Could you check a few things on this model? Use its own coordinates, in mm. Face numbers are marked on the shaded views. A direction names the side the tool comes from. Give positions to 0.01 mm unless a question says otherwise; leave off trailing zeros. Loops run counter-clockwise (first coordinate to the right, second up) from the corner with the lowest first, then second, coordinate; pieces in that order, holes last. Notation, with made-up numbers: (79, -27) -> (105, -27) arc R33 ccw to (105, 1) -> close; hole circle Ø6 at (-5, 69.25). An arc over 180 degrees is marked (long way). Write each question's results on one line, items separated by ' | '. Start each with the question number.
Q1. We'd pull the mould along Z, two halves only. Please class the marked faces 3, 4 and 5: released by +Z, released by -Z, zero draft, split by the parting line, or undercut.
Q2. If we section it at D-D, the plane x = 4: List the corners of the cut face in (y, z) for me.
Q3. If we section it at C-C, the plane x = 0: List the corners of the cut face in (y, z) for me.
Q4. Which directions (+Z, -Z, +X, -X, +Y, -Y) give clear straight access to the entire face, cutting with the end or side of a thin tool? Please do the marked faces 1 and 2.
Q5. If I drill on line 1 along Y through (x, z) = (6.25, 0); line 2 along Z through (x, y) = (2.75, 3), over which ranges is the centre line in solid material (lowest first)?
Q6. If we section it at A-A, the plane z = 0: List the corners of the cut face in (x, y) for me, plus the area to 3 significant figures.
from build123d import *

# Parameters (mm, degrees)
SKETCH1_W              = 25
SKETCH1_H              = 25
BOSS_EXTRUDE1_DEPTH    = 3
M14_TAPPED_HOLE1_D     = 12
M14_TAPPED_HOLE1_DEPTH = 34
M14_TAPPED_HOLE1_TIP   = 3.605163714
SKETCH5_R              = 11
SKETCH5_R_2            = 7.05
BOSS_EXTRUDE2_DEPTH    = 7
CUT_EXTRUDE1_START     = -1
SKETCH6_R              = 11
SKETCH6_R_2            = 8.7
CUT_EXTRUDE1_DEPTH     = 1
CHAMFER1_SIZE          = 4


with BuildPart() as part:
    # Sketch1 → Boss-Extrude1 (new, symmetric)
    with BuildSketch(Plane(origin=(0, 0, 0), x_dir=(0, 0, -1), z_dir=(1, 0, 0))):
        Rectangle(SKETCH1_W, SKETCH1_H)
    extrude(amount=BOSS_EXTRUDE1_DEPTH, both=True)

    # M14 Tapped Hole1
    with Locations(Plane.ZY.offset(3)):
        with Locations((0, 0)):
            Hole(M14_TAPPED_HOLE1_D / 2, depth=M14_TAPPED_HOLE1_DEPTH)
            with Locations((0, 0, -(M14_TAPPED_HOLE1_DEPTH + M14_TAPPED_HOLE1_TIP / 2))):  # 118° drill point
                Cone(0, M14_TAPPED_HOLE1_D / 2, M14_TAPPED_HOLE1_TIP, mode=Mode.SUBTRACT)

    # Sketch5 → Boss-Extrude2 (add)
    with BuildSketch(Plane(origin=(3, 0, 0), x_dir=(0, 0, -1), z_dir=(1, 0, 0))):
        Circle(SKETCH5_R)
        Circle(SKETCH5_R_2, mode=Mode.SUBTRACT)
    extrude(amount=BOSS_EXTRUDE2_DEPTH)

    # Sketch6 → Cut-Extrude1 (cut)
    with BuildSketch(Plane(origin=(10, 0, 0), x_dir=(0, 0, -1), z_dir=(1, 0, 0)).offset(CUT_EXTRUDE1_START)):
        Circle(SKETCH6_R)
        Circle(SKETCH6_R_2, mode=Mode.SUBTRACT)
    extrude(amount=CUT_EXTRUDE1_DEPTH, mode=Mode.SUBTRACT)

    # Chamfer1
    chamfer1_edges = [part.edges().sort_by_distance(p)[0] for p in [
        (0, -12.5, -12.5),
        (0, -12.5, 12.5),
        (0, 12.5, 12.5),
        (0, 12.5, -12.5),
    ]]
    chamfer(chamfer1_edges, length=CHAMFER1_SIZE)


solid = part.part
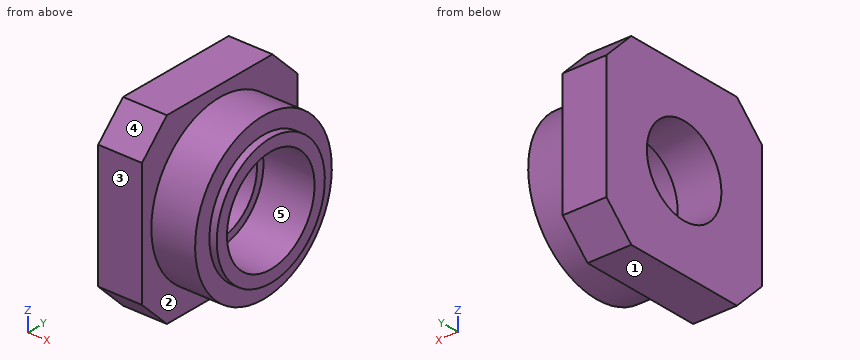
Final values:
1) face 3: zero draft | face 4: released by +Z | face 5: undercut
2) outline: circle Ø22 at (0, 0); hole circle Ø14.1 at (0, 0)
3) outline: (-12.5, -8.5) -> (-8.5, -12.5) -> (8.5, -12.5) -> (12.5, -8.5) -> (12.5, 8.5) -> (8.5, 12.5) -> (-8.5, 12.5) -> (-12.5, 8.5) -> close; hole circle Ø12 at (0, 0)
4) face 1: -Z, +X, -X, +Y, -Y | face 2: +X
5) line 1: y = -11 to -7.05, 7.05 to 11 | line 2: z = -12.5 to -5.2, 5.2 to 12.5
6) outline: (-3, -12.5) -> (3, -12.5) -> (3, -11) -> (9, -11) -> (9, -8.7) -> (10, -8.7) -> (10, -7.05) -> (3, -7.05) -> (3, -6) -> (-3, -6) -> close; (-3, 6) -> (3, 6) -> (3, 7.05) -> (10, 7.05) -> (10, 8.7) -> (9, 8.7) -> (9, 11) -> (3, 11) -> (3, 12.5) -> (-3, 12.5) -> close | area: 129 mm²
